Here's how the part is built. I have some questions about the finished solid (model axes, mm). Give positions to 0.01 mm unless a question says otherwise; leave off trailing zeros. Write each loop counter-clockwise with the first axis right and the second up, starting at its lowest first coordinate (ties: lowest second). Pieces come first, ordered by that corner, then holes. Notation, with made-up numbers: (4.25, -34.5) -> (24.25, -34.5) arc R24 cw to (24.25, -17.5) -> close; hole circle Ø9 at (27.25, 80.5). An arc over 180 degrees is marked (long way). Return JSON: item names as keys, results as strings.
from build123d import *

# Parameters (mm, degrees)
BOSS_EXTRUDE1_DEPTH = 550


with BuildPart() as part:
    # Sketch1 → Boss-Extrude1 (new body)
    with BuildSketch(Plane.XY):
        with BuildLine():
            Line((6, 0), (44, 0))
            ThreePointArc((44, 0), (48.242640687, 1.757359313), (50, 6))
            Line((50, 6), (50, 44))
            ThreePointArc((50, 44), (48.242640687, 48.242640687), (44, 50))
            Line((44, 50), (6, 50))
            ThreePointArc((6, 50), (1.757359313, 48.242640687), (0, 44))
            Line((0, 44), (0, 6))
            ThreePointArc((0, 6), (1.757359313, 1.757359313), (6, 0))
        make_face()
        with BuildLine():
            Line((6, 45), (44, 45))
            ThreePointArc((44, 45), (44.707106781, 44.707106781), (45, 44))
            Line((45, 44), (45, 6))
            ThreePointArc((45, 6), (44.707106781, 5.292893219), (44, 5))
            Line((44, 5), (6, 5))
            ThreePointArc((6, 5), (5.292893219, 5.292893219), (5, 6))
            Line((5, 6), (5, 44))
            ThreePointArc((5, 44), (5.292893219, 44.707106781), (6, 45))
        make_face(mode=Mode.SUBTRACT)
    extrude(amount=BOSS_EXTRUDE1_DEPTH)


solid = part.part
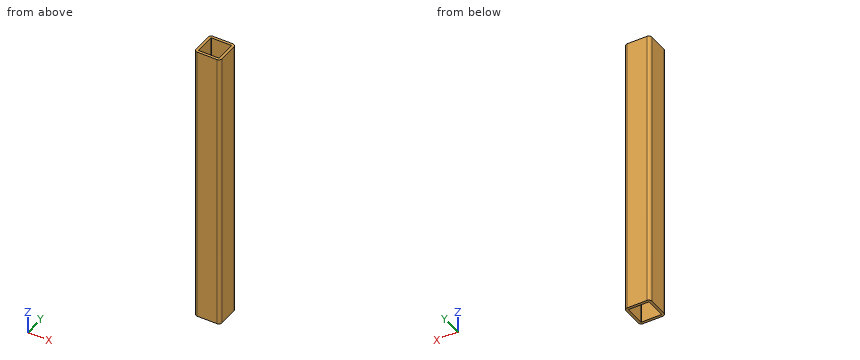
1. Suppose I cut it at A-A, the plane x = 19. List the corners of the cut face in (y, z) for me, and give its area (3 significant figures).
Taken from the geometry:
{"outline": "(0, 0) -> (5, 0) -> (5, 550) -> (0, 550) -> close; (45, 0) -> (50, 0) -> (50, 550) -> (45, 550) -> close", "area": "5,500 mm²"}
2. If I drill on line 1 (X direction, y = 15.5, z = 178.5); line 2 (X direction, y = 3.5, z = 257), over which ranges is the centre line in solid material (lowest first)? Write a range as [from, to].
Taken from the geometry:
{"line 1": "x = [0, 5], [45, 50]", "line 2": "x = [0.55, 49.45]"}
3. Suppose I cut it at C-C, the plane z = 36. List the corners of the cut face in (x, y) for me, and give its area (3 significant figures).
Taken from the geometry:
{"outline": "(0, 6) arc R6 ccw to (6, 0) -> (44, 0) arc R6 ccw to (50, 6) -> (50, 44) arc R6 ccw to (44, 50) -> (6, 50) arc R6 ccw to (0, 44) -> close; hole (5, 6) arc R1 ccw to (6, 5) -> (44, 5) arc R1 ccw to (45, 6) -> (45, 44) arc R1 ccw to (44, 45) -> (6, 45) arc R1 ccw to (5, 44) -> close", "area": "870 mm²"}
